Read the model definition and answer for the solid it produces. Units are mm, in the model's axes. A direction names the side the tool comes from. Round coordinates to 2 decimals unless told otherwise and drop trailing zeros. Order: outer loops, then holes, each group sorted by start corner. A loop starts at its lowest first (then second) coordinate and runs counter-clockwise, first axis right, second up. Notation, with made-up numbers: M 55.5,68 L 100.5,68 A20 cw 100.5,94 Z; hole C 8,68 d10. An arc over 180 degrees is marked long. Answer as CSV lines item,"result".
```python
from build123d import *

# Parameters (mm, degrees)
BASE_PROFILE_DEPTH     = 10
UPRIGHT_BLOCK_SKETCH_W = 30
UPRIGHT_BLOCK_SKETCH_H = 55
UPRIGHT_BLOCK_DEPTH    = 25
SLOTTED_ARM_DEPTH      = 15
THROUGH_HOLES_SKETCH_R = 5
THROUGH_HOLES_2X_DEPTH = 55


with BuildPart() as part:
    # Base Profile Sketch → Base Profile (new body)
    with BuildSketch(Plane.XY):
        Polygon((0, 0), (0, -55), (110, -55), (110, -35), (75, -35), (75, -42.5), (50, -42.5), (50, -12.5), (75, -12.5), (75, -20), (110, -20), (110, 0), align=None)
    extrude(amount=BASE_PROFILE_DEPTH)

    # Upright Block Sketch → Upright Block (add)
    with BuildSketch(Plane.XY.offset(10)):
        with Locations((15, -27.5)):
            Rectangle(UPRIGHT_BLOCK_SKETCH_W, UPRIGHT_BLOCK_SKETCH_H)
    extrude(amount=UPRIGHT_BLOCK_DEPTH)

    # Slotted Arm Sketch → Slotted Arm (add)
    with BuildSketch(Plane.XY.offset(10)):
        Polygon((30, 0), (30, -55), (95, -55), (95, -35), (75, -35), (75, -42.5), (50, -42.5), (50, -12.5), (75, -12.5), (75, -20), (95, -20), (95, 0), align=None)
    extrude(amount=SLOTTED_ARM_DEPTH)

    # Through Holes Sketch → Through Holes 2x (cut)
    with BuildSketch(Plane.XY.offset(35)):
        with Locations((15, -10)):
            Circle(THROUGH_HOLES_SKETCH_R)
        with Locations((15, -45)):
            Circle(THROUGH_HOLES_SKETCH_R)
    extrude(amount=-THROUGH_HOLES_2X_DEPTH, mode=Mode.SUBTRACT)


solid = part.part
```
Item 1: A cutting plane is placed at C-C, the plane y = -45. Determine the outline of the cut face in (x, z), and give its area (4 significant figures).
Ans:
outline,"M 0,0 L 10,0 L 10,35 L 0,35 Z; M 20,0 L 110,0 L 110,10 L 95,10 L 95,25 L 30,25 L 30,35 L 20,35 Z"
area,"2,475 mm2"
Item 2: A cutting plane is placed at B-B, the plane x = 100.5. Determine the outline of the cut face in (y, z).
Ans:
outline,"M -55,0 L -35,0 L -35,10 L -55,10 Z; M -20,0 L 0,0 L 0,10 L -20,10 Z"
Item 3: Determine the mould class of faces 1 (the face through (95, -45, 17)), 2 (the face through (89, -35, 10)), 3 (the face through (50, -28, 12)) for opening direction X: +X half, -X half, draft (parallel to the pull), parting line (faces both ways), or undercut.
Ans:
face 1,"+X half"
face 2,"draft"
face 3,"undercut"
Item 4: A cutting plane is placed at A-A, the plane z = 20.5. Determine the outline of the cut face in (x, y).
Ans:
outline,"M 0,-55 L 95,-55 L 95,-35 L 75,-35 L 75,-42.5 L 50,-42.5 L 50,-12.5 L 75,-12.5 L 75,-20 L 95,-20 L 95,0 L 0,0 Z; hole C 15,-45 d10; hole C 15,-10 d10"
Item 5: Find the intervals of material crossed by probe 1 along Y at (x, z) = (15, 17); probe 2 along Y at (x, z) = (79, 14); probe 3 along Y at (x, z) = (54.5, 2), in increasing order. Write a range as [from, to].
Ans:
probe 1,"[-55, -50], [-40, -15], [-5, 0]"
probe 2,"[-55, -35], [-20, 0]"
probe 3,"[-55, -42.5], [-12.5, 0]"
Item 6: A cutting plane is placed at D-D, the plane x = 15. Determine the outline of the cut face in (y, z).
Ans:
outline,"M -55,0 L -50,0 L -50,35 L -55,35 Z; M -40,0 L -15,0 L -15,35 L -40,35 Z; M -5,0 L 0,0 L 0,35 L -5,35 Z"
Item 7: A tool of negligible diameter and unlimited length cuts with its end or side. For faces 4 (the face through (44, 0, 13)), 5 (the face through (102, -45, 10)), 6 (the face through (63, -42.5, 12)), 7 (the face through (88, -20, 10)), from which of +Z, -Z, +X, -X, +Y, -Y can it reach the whole face along a straight path? Write none if from no direction.
Ans:
face 4,"+Z, -Z, +X, -X, +Y"
face 5,"+Z, +X, +Y, -Y"
face 6,"+Z, -Z"
face 7,"+Z, -Z, +X"
Item 8: Flat-ended cylindrical pins translate along their axes: pin 1 (8 mm diameter, centred on x = 15, y = -45, fed in from +Z); pin 2 (5 mm diameter, centred on y = -12.5, z = 27, fed in from +X); pin 3 (10 mm diameter, centred on y = -12, z = 31.5, fed in from +X); pin 4 (16.5 mm diameter, centred on x = 102, y = -14, fed in from +Z). Find the tip coordinate at first contact, or state that the pin passes through.
Ans:
pin 1,"through"
pin 2,"x = 95"
pin 3,"x = 30"
pin 4,"z = 25"
